Source: CAD feature listing. Evaluate the final solid. Frame: model axes, mm. A direction names the side the tool comes from. Round coordinates to 2 decimals unless told otherwise and drop trailing zeros. Write each loop counter-clockwise with the first axis right and the second up, starting at its lowest first coordinate (ties: lowest second). Pieces come first, ordered by that corner, then holes. Notation, with made-up numbers: M 78.25,88 L 137.25,88 A19 ccw 137.25,92 Z; hole C -7.5,26 d1. An arc over 180 degrees is marked long. Answer in a Markdown table with one row per item. Add a question column.
Item 1: Cut plane C-C on x = -133.5. Return loops of the section in (y, z).
Item 2: Cut plane D-D on z = 12. Give the number of separate pieces and of enclosed holes in the cut face, and give its area (3 significant figures).
Item 3: Set-up query: faces 5 (the face through (164.28, 265.49, -0.28)), 6 (the face through (126.014, 284.297, 0.28)), 7 (the face through (-42.5, 84, 0)). Return all of +Z, -Z, +X, -X, +Y, -Y with unobstructed straight access to the full face (end or side cutting, diameter ignored); none if empty.
Item 4: Cut plane B-B on x = -230.5. Return loops of the section in (y, z), and give its area (3 significant figures).
Item 5: Cut plane A-A on y = 119. Return loops of the section in (x, z).
Item 6: Material intervals for probe 1 along X at (y, z) = (82, -12.5); probe 2 along Y at (x, z) = (-223, -14.5); probe 3 along X at (y, z) = (244.5, -2), sorted ascending.
Item 7: Contact query for flat-ended pins moving along their axis: pin 1 (10 mm diameter, centred on x = 79, z = 15.5, fed in from +Y); pin 2 (12 mm diameter, centred on x = -124, z = -5, fed in from +Y). Output: stop coordinate, or through.
Item 8: Mould query, pull axis Y, two halves, no side actions, for faces 1 (the face through (212.01, 170.72, -0.28)), 2 (the face through (-320, 147, 0)), 3 (the face through (211.78, 49.51, 0.28)), 4 (the face through (180, 0, 0)). Classes: released by +Y, released by -Y, zero draft, split by the parting line, or undercut.
from build123d import *

# Parameters (mm, degrees)
SKETCH1_W            = 120
SKETCH1_H            = 50
BOSS_EXTRUDE1_DEPTH  = 20
FILLET1_R            = 15
SKETCH2_W            = 75
SKETCH2_H            = 130
CUT_EXTRUDE1_DEPTH   = 433.319326424
FILLET2_R            = 15
FILLET2_OF_MIRROR1_R = 15


with BuildPart() as part:
    # Sketch1 → Boss-Extrude1 (new, symmetric)
    with BuildSketch(Plane.XY):
        with BuildLine():
            Line((42.5, 150), (42.5, 20))
            ThreePointArc((42.5, 20), (48.357864376, 5.857864376), (62.5, 0))
            Line((62.5, 0), (300, 0))
            ThreePointArc((300, 0), (314.142135624, 5.857864376), (320, 20))
            Line((320, 20), (320, 270))
            ThreePointArc((320, 270), (314.142135624, 284.142135624), (300, 290))
            Line((300, 290), (140, 290))
            ThreePointArc((140, 290), (125.857864376, 284.142135624), (120, 270))
            Line((120, 270), (120, 240))
            ThreePointArc((120, 240), (114.142135624, 225.857864376), (100, 220))
            Line((100, 220), (-100, 220))
            ThreePointArc((-100, 220), (-114.142135624, 225.857864376), (-120, 240))
            Line((-120, 240), (-120, 270))
            ThreePointArc((-120, 270), (-125.857864376, 284.142135624), (-140, 290))
            Line((-140, 290), (-300, 290))
            ThreePointArc((-300, 290), (-314.142135624, 284.142135624), (-320, 270))
            Line((-320, 270), (-320, 20))
            ThreePointArc((-320, 20), (-314.142135624, 5.857864376), (-300, 0))
            Line((-300, 0), (-62.5, 0))
            ThreePointArc((-62.5, 0), (-48.357864376, 5.857864376), (-42.5, 20))
            Line((-42.5, 20), (-42.5, 150))
            ThreePointArc((-42.5, 150), (0, 192.5), (42.5, 150))
        make_face()
        with Locations((-220, 245)):
            Rectangle(SKETCH1_W, SKETCH1_H, mode=Mode.SUBTRACT)
        with Locations((220, 245)):
            Rectangle(SKETCH1_W, SKETCH1_H, mode=Mode.SUBTRACT)
    extrude(amount=BOSS_EXTRUDE1_DEPTH, both=True)

    # Fillet1
    fillet1_edges = [part.edges().sort_by_distance(p)[0] for p in [
        (-160, 220, 0),
        (-160, 270, 0),
        (-280, 270, 0),
        (-280, 220, 0),
        (280, 220, 0),
        (280, 270, 0),
        (160, 270, 0),
        (160, 220, 0),
    ]]
    fillet(fillet1_edges, radius=FILLET1_R)

    # Sketch2 → Cut-Extrude1 (cut, symmetric)
    with BuildSketch(Plane.XY):
        with Locations((-245, 110)):
            Rectangle(SKETCH2_W, SKETCH2_H)
        with Locations((-125, 110)):
            Rectangle(SKETCH2_W, SKETCH2_H)
    cut_extrude1 = extrude(amount=CUT_EXTRUDE1_DEPTH, both=True, mode=Mode.SUBTRACT)

    # Fillet2
    fillet2_edges = [part.edges().sort_by_distance(p)[0] for p in [
        (-207.5, 175, 0),
        (-207.5, 45, 0),
        (-282.5, 45, 0),
        (-282.5, 175, 0),
        (-87.5, 175, 0),
        (-87.5, 45, 0),
        (-162.5, 45, 0),
        (-162.5, 175, 0),
    ]]
    fillet(fillet2_edges, radius=FILLET2_R)

    # Mirror1: Cut-Extrude1 across plane
    add(cut_extrude1.mirror(Plane(origin=(0, 0, 0), x_dir=(0, 0, 1), z_dir=(1, 0, 0))), mode=Mode.SUBTRACT)

    # Fillet2 of Mirror1
    fillet2_of_mirror1_edges = [part.edges().sort_by_distance(p)[0] for p in [
        (207.5, 175, 0),
        (207.5, 45, 0),
        (282.5, 45, 0),
        (282.5, 175, 0),
        (87.5, 175, 0),
        (87.5, 45, 0),
        (162.5, 45, 0),
        (162.5, 175, 0),
    ]]
    fillet(fillet2_of_mirror1_edges, radius=FILLET2_OF_MIRROR1_R)


solid = part.part
Results below:
| question | item | result |
|---|---|---|
| 1 | outline | M 0,-20 L 45,-20 L 45,20 L 0,20 Z; M 175,-20 L 288.91,-20 L 288.91,20 L 175,20 Z |
| 2 | separate pieces | 1 |
| 2 | enclosed holes | 6 |
| 2 | area | 103,000 mm2 |
| 3 | face 5 | +Z, -Z |
| 3 | face 6 | +Z, -Z, +Y |
| 3 | face 7 | +Z, -Z, -Y |
| 4 | outline | M 0,-20 L 45,-20 L 45,20 L 0,20 Z; M 175,-20 L 220,-20 L 220,20 L 175,20 Z; M 270,-20 L 290,-20 L 290,20 L 270,20 Z |
| 4 | area | 4,400 mm2 |
| 5 | outline | M -320,-20 L -282.5,-20 L -282.5,20 L -320,20 Z; M -207.5,-20 L -162.5,-20 L -162.5,20 L -207.5,20 Z; M -87.5,-20 L -42.5,-20 L -42.5,20 L -87.5,20 Z; M 42.5,-20 L 87.5,-20 L 87.5,20 L 42.5,20 Z; M 162.5,-20 L 207.5,-20 L 207.5,20 L 162.5,20 Z; M 282.5,-20 L 320,-20 L 320,20 L 282.5,20 Z |
| 6 | probe 1 | -320 to -282.5, -207.5 to -162.5, -87.5 to -42.5, 42.5 to 87.5, 162.5 to 207.5, 282.5 to 320 |
| 6 | probe 2 | 0 to 45, 175 to 220, 270 to 290 |
| 6 | probe 3 | -320 to -280, -160 to -120, 120 to 160, 280 to 320 |
| 7 | pin 1 | y = 220 |
| 7 | pin 2 | y = 287.32 |
| 8 | face 1 | undercut |
| 8 | face 2 | zero draft |
| 8 | face 3 | undercut |
| 8 | face 4 | released by -Y |
